```python
from build123d import *

# Parameters (mm, degrees)
END_SLOT_CUT_DEPTH      = 51.539588475
END_SLOT_CUT_DEPTH_BACK = 51.539588475
END_SLOT_PROFILE_W      = 5
END_SLOT_PROFILE_H      = 4


with BuildPart() as part:
    # Bushing Revolve Profile → Stepped Bushing Body (revolve)
    with BuildSketch(Plane.XY, mode=Mode.PRIVATE) as stepped_bushing_body_sk:
        with BuildLine():
            Line((0, 0), (0, -1))
            ThreePointArc((0, -1), (0.292893219, -1.707106781), (1, -2))
            Line((1, -2), (12, -2))
            Line((12, -2), (18, -8))
            Line((18, -8), (27.5, -8))
            Line((27.5, -8), (27.5, -7))
            ThreePointArc((27.5, -7), (27.792893219, -6.292893219), (28.5, -6))
            Line((28.5, -6), (32.5, -6))
            ThreePointArc((32.5, -6), (33.207106781, -6.292893219), (33.5, -7))
            Line((33.5, -7), (33.5, -8))
            Line((33.5, -8), (40.5, -8))
            ThreePointArc((40.5, -8), (41.207106781, -7.707106781), (41.5, -7))
            Line((41.5, -7), (41.5, 0))
            Line((41.5, 0), (0, 0))
        make_face()
    revolve(stepped_bushing_body_sk.sketch.rotate(Axis((-18.754371045, 8, 0), (1, 0, 0)), 270), axis=Axis((-18.754371045, 8, 0), (1, 0, 0)))

    # End Slot Profile → End Slot Cut (cut, two sides: drawn at the far end of the back side and taken through both)
    with BuildSketch(Plane.XY.offset(-END_SLOT_CUT_DEPTH_BACK)):
        with Locations((2.5, 8)):
            Rectangle(END_SLOT_PROFILE_W, END_SLOT_PROFILE_H)
    extrude(amount=END_SLOT_CUT_DEPTH + END_SLOT_CUT_DEPTH_BACK, mode=Mode.SUBTRACT)


solid = part.part
```
Geometry check sheet. Reference: the model listing, model coordinates, mm. A direction names the side the tool comes from. Coordinates: 2 decimals unless noted, no trailing zeros. Order: outer loops, then holes, each group sorted by start corner. A loop starts at its lowest first (then second) coordinate and runs counter-clockwise, first axis right, second up. Notation, with made-up numbers: (40.5, 64) - (68.5, 64) arc R21 ccw to (68.5, 83) - close; hole circle Ø10 at (-36.5, -1.75). An arc over 180 degrees is marked (long way). Answer as a JSON object with one key per item and string values. Group by question number.
Item 1: Sectioned sample at A-A, the plane y = 8. Record the cut outline in (x, z).
Item 2: Sectioned sample at C-C, the plane x = 24.5. Record the cut outline in (y, z).
Item 3: Depth check by flat-ended pin: pin 1 Ø12 at (x, y) = (36, 20) entering from +Z; pin 2 Ø1 at (x, y) = (6.5, -4) entering from -Z; pin 3 Ø1.5 at (x, z) = (33.5, 2.5) entering from -Y; pin 4 Ø2.5 at (y, z) = (8, -9) entering from -X. Enter the tip coordinate at first touch or a pass-through.
Item 4: Draft check along Y on faces 4 (the face through (0, 16.3, 0.7)), 5 (the face through (6.58, 5, 9.54)), 6 (the face through (20.46, 11.06, 7.39)). Enter one of: +Y half, -Y half, draft (parallel to the pull), parting line (faces both ways), or undercut.
Item 5: Scan lines: probe 1 along Y at (x, z) = (22.5, 0); probe 2 along Y at (x, z) = (32, 0); probe 3 along X at (y, z) = (16, -12). Record each from-to range of solid material in increasing order.
Item 6: Sectioned sample at D-D, the plane x = 7. Record the cut outline in (y, z), and give its area (3 significant figures).
Item 7: Tool access check on faces 1 (the face through (2, 6, 9)), 2 (the face through (30.53, 21.67, -3.03)), 3 (the face through (22.816, -7.864, -2.083)). Record the directions out of +Z, -Z, +X, -X, +Y, -Y that give a thin tool (end or side, any length) a straight path to the whole face; none if there is none.
Item 8: Sectioned sample at B-B, the plane z = 0. Record the cut outline in (x, y).
Resolved:
{
 "1": {"outline": "(5, -10) - (12, -10) - (18, -16) - (27.5, -16) - (27.5, -15) arc R1 cw to (28.5, -14) - (32.5, -14) arc R1 cw to (33.5, -15) - (33.5, -16) - (40.5, -16) arc R1 ccw to (41.5, -15) - (41.5, -8) - (5, -8) - close; (5, 8) - (41.5, 8) - (41.5, 15) arc R1 ccw to (40.5, 16) - (33.5, 16) - (33.5, 15) arc R1 cw to (32.5, 14) - (28.5, 14) arc R1 cw to (27.5, 15) - (27.5, 16) - (18, 16) - (12, 10) - (5, 10) - close"},
 "2": {"outline": "circle Ø32 at (8, 0); hole circle Ø16 at (8, 0)"},
 "3": {"pin 1": "z = 14.83", "pin 2": "through", "pin 3": "y = -7.9", "pin 4": "x = 5"},
 "4": {"face 4": "draft", "face 5": "parting line", "face 6": "undercut"},
 "5": {"probe 1": "-8 to 0, 16 to 24", "probe 2": "-6 to 0, 16 to 22", "probe 3": "16.42 to 27.68, 33.32 to 41.5"},
 "6": {"outline": "circle Ø20 at (8, 0); hole circle Ø16 at (8, 0)", "area": "113 mm^2"},
 "7": {"face 1": "+Z, -Z, -X", "face 2": "none", "face 3": "+X, -X"},
 "8": {"outline": "(0, -1) arc R1 ccw to (1, -2) - (12, -2) - (18, -8) - (27.5, -8) - (27.5, -7) arc R1 cw to (28.5, -6) - (32.5, -6) arc R1 cw to (33.5, -7) - (33.5, -8) - (40.5, -8) arc R1 ccw to (41.5, -7) - (41.5, 0) - (0, 0) - close; (0, 16) - (41.5, 16) - (41.5, 23) arc R1 ccw to (40.5, 24) - (33.5, 24) - (33.5, 23) arc R1 cw to (32.5, 22) - (28.5, 22) arc R1 cw to (27.5, 23) - (27.5, 24) - (18, 24) - (12, 18) - (1, 18) arc R1 ccw to (0, 17) - close"}
}
